Can you work these out from the drawing? Everything is in mm from the part's minimum corner. Round coordinates to 2 decimals unless told otherwise and drop trailing zeros. Order: outer loops, then holes, each group sorted by start corner. A loop starts at its lowest first (then second) coordinate and runs counter-clockwise, first axis right, second up. Notation, with made-up numbers: (24.25, 56) - (74.25, 56) arc R19 ccw to (74.25, 75) - close; hole circle Ø11 at (-15.5, -6.5). An arc over 180 degrees is marked (long way). Answer as a JSON object with one key per item and string values.
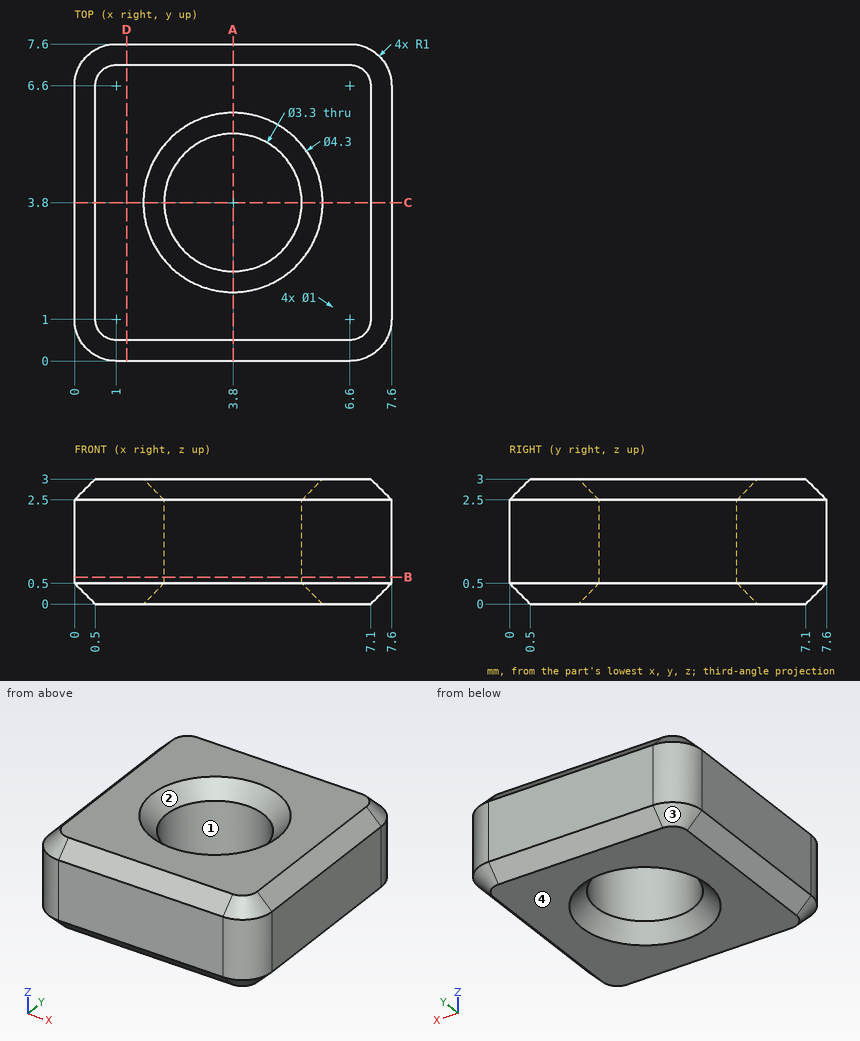
1. Imagine slicing it at D-D (x = 1.25). List the corners of the cut face in (y, z) for me, plus the area to 3 significant figures.
Responses:
{"outline": "(0, 0.5) - (0.5, 0) - (7.1, 0) - (7.6, 0.5) - (7.6, 2.5) - (7.1, 3) - (0.5, 3) - (0, 2.5) - close", "area": "22.3 mm2"}
2. If I drill on L1, parallel to Y at x = 3.8, z = 1.25; L2, parallel to X at y = 2.5, z = 2.3; L3, parallel to Y at x = 2.25, z = 2.7, over which ranges is the centre line in solid material (lowest first)? Write a range as [from, to].
Responses:
{"L1": "[0, 2.15], [5.45, 7.6]", "L2": "[0, 2.78], [4.82, 7.6]", "L3": "[0.2, 2.79], [4.81, 7.4]"}
3. Imagine slicing it at A-A (x = 3.8). List the corners of the cut face in (y, z) for me.
Responses:
{"outline": "(0, 0.5) - (0.5, 0) - (1.65, 0) - (2.15, 0.5) - (2.15, 2.5) - (1.65, 3) - (0.5, 3) - (0, 2.5) - close; (5.45, 0.5) - (5.95, 0) - (7.1, 0) - (7.6, 0.5) - (7.6, 2.5) - (7.1, 3) - (5.95, 3) - (5.45, 2.5) - close"}
4. For P1, Ø4, axis at x = 3.8, y = 3.8, coming from the +Z side, with a flat end and sliding along its axis, tell me the tip position at first contact or that it passes through.
Responses:
{"P1": "z = 2.85"}
5. Thinking about a two-plate mould opening in Y: for the marked faces 1, 2, 3 and 4, which applies, pulls with the +Y half, pulls with the -Y half, needs draft (parallel to the pull), parting line crosses it, or undercut?
Responses:
{"face 1": "undercut", "face 2": "undercut", "face 3": "pulls with the +Y half", "face 4": "needs draft"}
6. Imagine slicing it at B-B (z = 0.65). List the corners of the cut face in (x, y) for me, plus the area to 3 significant figures.
Responses:
{"outline": "(0, 1) arc R1 ccw to (1, 0) - (6.6, 0) arc R1 ccw to (7.6, 1) - (7.6, 6.6) arc R1 ccw to (6.6, 7.6) - (1, 7.6) arc R1 ccw to (0, 6.6) - close; hole circle Ø3.3 at (3.8, 3.8)", "area": "48.3 mm2"}
